Read the model definition and answer for the solid it produces. Units are mm, in the model's axes. Coordinates: 2 decimals unless noted, no trailing zeros. Write each loop counter-clockwise with the first axis right and the second up, starting at its lowest first coordinate (ties: lowest second). Pieces come first, ordered by that corner, then holes.
(1) The part is cut by section A-A, the plane z = 31.5. Determine the outline of the cut face in (x, y), and give its area (3 significant figures).
(2) Straight lines are drawn through the part: line 1 along X through (y, z) = (0.25, 13.5); line 2 along Y through (x, z) = (0, 1); line 3 along Y through (x, z) = (-1, 8.5). For each, find the intervals that lie inside material, in ascending order.
(3) Given pin 1 (3.5 mm diameter, centred on x = 0, y = 0, fed in from -Z); pin 2 (1 mm diameter, centred on x = 0.5, z = 105.5, fed in from -Y); pin 3 (1.5 mm diameter, centred on y = 1, z = 23, fed in from -X); pin 4 (2.5 mm diameter, centred on y = -0.5, z = -28.5, fed in from +X), each flat-ended and moving along its own axis, determine where each tip first touches the part or whether it passes through.
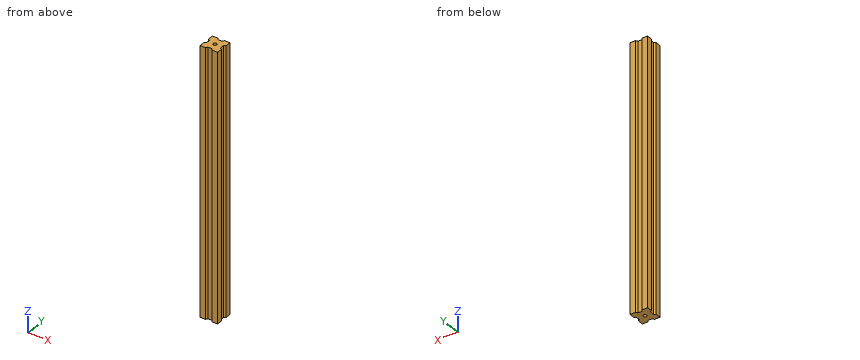
```python
from build123d import *

# Parameters (mm, degrees)
SKETCH_1_W               = 20
SKETCH_1_H               = 20
SKETCH_1_R               = 1.94442565
EXTRUDE_1_DEPTH          = 150
CUT_EXTRUDE_1_DEPTH      = 301.333148354
PATTERN_CIRCULAR_1_COUNT = 4


with BuildPart() as part:
    # 草图1 → 凸台-拉伸1 (new, symmetric)
    with BuildSketch(Plane.XY):
        Rectangle(SKETCH_1_W, SKETCH_1_H)
        Circle(SKETCH_1_R, mode=Mode.SUBTRACT)
    extrude(amount=EXTRUDE_1_DEPTH, both=True)

    # 草图2 → 切除-拉伸1 (cut, symmetric)
    with BuildSketch(Plane.XY.offset(150)):
        Polygon((-32.933615203, 60.643738676), (-3.694439046, 10), (-2.5, 7.931170886), (2.5, 7.931170886), (3.694439046, 10), (32.933615203, 60.643738676), (32.933615203, 177.600443305), (-32.933615203, 177.600443305), align=None)
    cut_extrude_1 = extrude(amount=CUT_EXTRUDE_1_DEPTH, both=True, mode=Mode.SUBTRACT)

    # 阵列(圆周)1: 切除-拉伸1 ×4 about axis
    pattern_circular_1_axis = Axis((0, 0, 150), (0, 0, -1))
    for i in range(1, PATTERN_CIRCULAR_1_COUNT):
        add(cut_extrude_1.rotate(pattern_circular_1_axis, i * 360 / PATTERN_CIRCULAR_1_COUNT), mode=Mode.SUBTRACT)


solid = part.part
```
Computed:
1. outline: (-10, -10) - (-3.69, -10) - (-2.5, -7.93) - (2.5, -7.93) - (3.69, -10) - (10, -10) - (10, -3.69) - (7.93, -2.5) - (7.93, 2.5) - (10, 3.69) - (10, 10) - (3.69, 10) - (2.5, 7.93) - (-2.5, 7.93) - (-3.69, 10) - (-10, 10) - (-10, 3.69) - (-7.93, 2.5) - (-7.93, -2.5) - (-10, -3.69) - close; hole circle Ø3.89 at (0, 0)
1. area: 337 mm2
2. line 1: x = -7.93 to -1.93, 1.93 to 7.93
2. line 2: y = -7.93 to -1.94, 1.94 to 7.93
2. line 3: y = -7.93 to -1.67, 1.67 to 7.93
3. pin 1: passes through
3. pin 2: stops at y = -7.93
3. pin 3: stops at x = -7.93
3. pin 4: stops at x = 7.93
